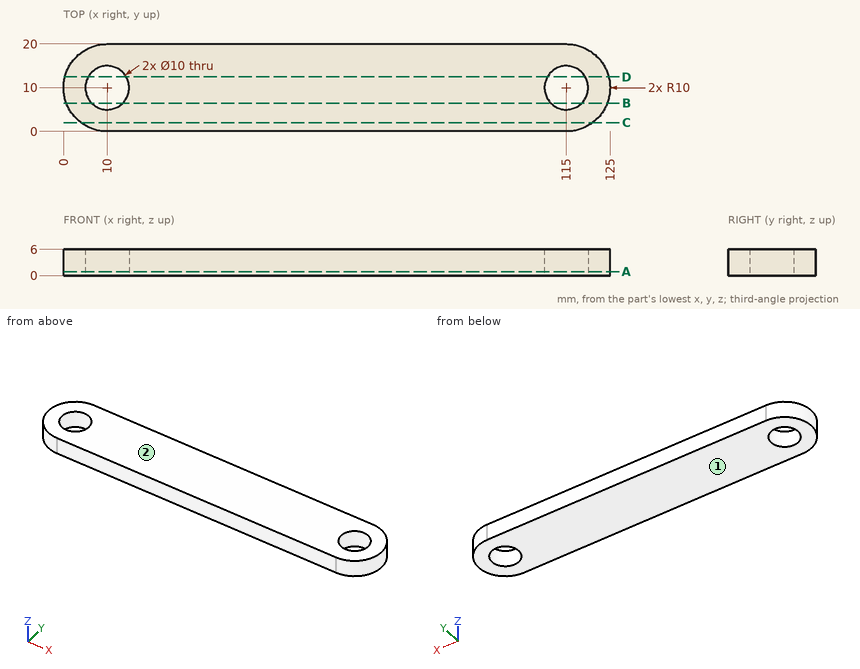
Drawing for the job (mm, zero at the part's lowest x, y, z). Coordinates: 2 decimals unless noted, no trailing zeros. Order: outer loops, then holes, each group sorted by start corner. A loop starts at its lowest first (then second) coordinate and runs counter-clockwise, first axis right, second up. Notation, with made-up numbers: (-1.5, 69.25) -> (16.5, 69.25) arc R24 ccw to (16.5, 96.25) -> close; hole circle Ø3 at (17.25, 12). An arc over 180 degrees is marked (long way). Return JSON: item names as keys, results as strings.
Item 1: Wall check: line 1 along Y through (x, z) = (10, 4.4); line 2 along X through (y, z) = (8.75, 2.8); line 3 along X through (y, z) = (9, 1.8). Give the ranges that are in metal, low to high. Write a range as from..to.
Model answer:
{"line 1": "y = 0..5, 15..20", "line 2": "x = 0.08..5.16, 14.84..110.16, 119.84..124.92", "line 3": "x = 0.05..5.1, 14.9..110.1, 119.9..124.95"}
Item 2: Slice it at C-C (y = 2). Write the cut outline in (x, z).
Model answer:
{"outline": "(4, 0) -> (121, 0) -> (121, 6) -> (4, 6) -> close"}
Item 3: Slice it at D-D (y = 12.5). Write the cut outline in (x, z).
Model answer:
{"outline": "(0.32, 0) -> (5.67, 0) -> (5.67, 6) -> (0.32, 6) -> close; (14.33, 0) -> (110.67, 0) -> (110.67, 6) -> (14.33, 6) -> close; (119.33, 0) -> (124.68, 0) -> (124.68, 6) -> (119.33, 6) -> close"}
Item 4: Slice it at A-A (z = 0.95). Write the cut outline in (x, y), then the cut area to 3 significant figures.
Model answer:
{"outline": "(10, 0) -> (115, 0) arc R10 ccw to (115, 20) -> (10, 20) arc R10 ccw to start; hole circle Ø10 at (10, 10); hole circle Ø10 at (115, 10)", "area": "2,260 mm²"}
Item 5: Pin check, flat tip, straight feed: P1, Ø1, axis at y = 14, z = 1.5, coming from the -X side. Stop position of the tip, or through.
Model answer:
{"P1": "stops at x = 0.63"}
Item 6: Mould opens along Z. For the marked faces 1 and 2 say: pulls with the +Z half, pulls with the -Z half, needs draft (parallel to the pull), parting line crosses it, or undercut.
Model answer:
{"face 1": "pulls with the -Z half", "face 2": "pulls with the +Z half"}
Item 7: Slice it at B-B (y = 6.5). Write the cut outline in (x, z), then the cut area to 3 significant figures.
Model answer:
{"outline": "(0.63, 0) -> (6.43, 0) -> (6.43, 6) -> (0.63, 6) -> close; (13.57, 0) -> (111.43, 0) -> (111.43, 6) -> (13.57, 6) -> close; (118.57, 0) -> (124.37, 0) -> (124.37, 6) -> (118.57, 6) -> close", "area": "657 mm²"}
